```python
from build123d import *

# Parameters (mm, degrees)
BOSS_EXTRUDE1_DEPTH = 16
SKETCH2_R           = 1
CUT_EXTRUDE1_DEPTH  = 16


with BuildPart() as part:
    # Sketch1 → Boss-Extrude1 (new body)
    with BuildSketch(Plane.XY):
        with BuildLine():
            Line((0, 0), (4, 0))
            ThreePointArc((4, 0), (5.414213562, 0.585786438), (6, 2))
            Line((6, 2), (6, 38))
            ThreePointArc((6, 38), (6.585786438, 39.414213562), (8, 40))
            Line((8, 40), (44, 40))
            ThreePointArc((44, 40), (45.414213562, 39.414213562), (46, 38))
            Line((46, 38), (46, 2))
            ThreePointArc((46, 2), (46.585786438, 0.585786438), (48, 0))
            Line((48, 0), (52, 0))
            Line((52, 0), (52, 1.5))
            Line((52, 1.5), (48, 1.5))
            ThreePointArc((48, 1.5), (47.646446609, 1.646446609), (47.5, 2))
            Line((47.5, 2), (47.5, 38))
            ThreePointArc((47.5, 38), (46.474873734, 40.474873734), (44, 41.5))
            Line((44, 41.5), (8, 41.5))
            ThreePointArc((8, 41.5), (5.525126266, 40.474873734), (4.5, 38))
            Line((4.5, 38), (4.5, 2))
            ThreePointArc((4.5, 2), (4.353553391, 1.646446609), (4, 1.5))
            Line((4, 1.5), (0, 1.5))
            Line((0, 1.5), (0, 0))
        make_face()
    extrude(amount=BOSS_EXTRUDE1_DEPTH)

    # Sketch2 → Cut-Extrude1 (cut)
    with BuildSketch(Plane(origin=(0, 1.5, 0), x_dir=(1, 0, 0), z_dir=(0, 1, 0))):
        with Locations(Location((50, -3, 0), (0, 0, 180))):
            Circle(SKETCH2_R)
        with Locations(Location((50, -13, 0), (0, 0, 180))):
            Circle(SKETCH2_R)
        with Locations(Location((2, -3, 0), (0, 0, 180))):
            Circle(SKETCH2_R)
        with Locations(Location((2, -13, 0), (0, 0, 180))):
            Circle(SKETCH2_R)
    extrude(amount=-CUT_EXTRUDE1_DEPTH, mode=Mode.SUBTRACT)


solid = part.part
```
Design review of the part built by this model. Coordinates are the model's own, in mm. A direction names the side the tool comes from. Coordinates: 2 decimals unless noted, no trailing zeros. Loops run counter-clockwise (first coordinate to the right, second up) from the corner with the lowest first, then second, coordinate; pieces in that order, holes last. Notation, with made-up numbers: (48, 78.25) -> (66, 78.25) arc R21 ccw to (66, 110.25) -> close; hole circle Ø1 at (68.5, -18.75). An arc over 180 degrees is marked (long way). Answer as a JSON object with one key per item and string values.
Q1. Clearance check with flat-ended pins moving along their axes: pin 1 Ø3 at (y, z) = (9, 11) entering from +X; pin 2 Ø6 at (x, z) = (5.5, 4) entering from +Y; pin 3 Ø2 at (x, z) = (1.5, 4.5) entering from +Y; pin 4 Ø5 at (x, z) = (26.5, 11) entering from -Y. State where each tip first meets the part, or that it passes through.
Answer block:
{"pin 1": "stops at x = 47.5", "pin 2": "stops at y = 41.5", "pin 3": "stops at y = 1.5", "pin 4": "stops at y = 40"}
Q2. Take a section at B-B on x = 2. Give the boundary of the cut face in (y, z), plus the area to 3 significant figures.
Answer block:
{"outline": "(0, 0) -> (1.5, 0) -> (1.5, 2) -> (0, 2) -> close; (0, 4) -> (1.5, 4) -> (1.5, 12) -> (0, 12) -> close; (0, 14) -> (1.5, 14) -> (1.5, 16) -> (0, 16) -> close", "area": "18.0 mm^2"}
Q3. Take a section at A-A on y = 5. Give the boundary of the cut face in (x, z), plus the area to 3 significant figures.
Answer block:
{"outline": "(4.5, 0) -> (6, 0) -> (6, 16) -> (4.5, 16) -> close; (46, 0) -> (47.5, 0) -> (47.5, 16) -> (46, 16) -> close", "area": "48.0 mm^2"}
Q4. Tool access review of faces 4 (the flat face through (50, 1.5, 8)), 5 (the flat face through (4.5, 20, 8)), 6 (the cylindrical face through (46.57, 0.6, 7.89)): name each direction out of +Z, -Z, +X, -X, +Y, -Y from which nothing blocks a thin tool from reaching the whole face with its end or side.
Answer block:
{"face 4": "+Z, -Z, +X, +Y", "face 5": "+Z, -Z, -X, +Y", "face 6": "+Z, -Z, -Y"}
Q5. Take a section at C-C on z = 3. Give the boundary of the cut face in (x, y), plus the area to 3 significant figures.
Answer block:
{"outline": "(0, 0) -> (1, 0) -> (1, 1.5) -> (0, 1.5) -> close; (3, 0) -> (4, 0) arc R2 ccw to (6, 2) -> (6, 38) arc R2 cw to (8, 40) -> (44, 40) arc R2 cw to (46, 38) -> (46, 2) arc R2 ccw to (48, 0) -> (49, 0) -> (49, 1.5) -> (48, 1.5) arc R0.5 cw to (47.5, 2) -> (47.5, 38) arc R3.5 ccw to (44, 41.5) -> (8, 41.5) arc R3.5 ccw to (4.5, 38) -> (4.5, 2) arc R0.5 cw to (4, 1.5) -> (3, 1.5) -> close; (51, 0) -> (52, 0) -> (52, 1.5) -> (51, 1.5) -> close", "area": "187 mm^2"}
Q6. To check wall thickness, follow L1, parallel to Z at x = 2, y = 1.25; L2, parallel to X at y = 13.5, z = 11.75; L3, parallel to Y at x = 37, z = 11.25. State the ranges of each line that lie inside material, in increasing order.
Answer block:
{"L1": "z = 0 to 2, 4 to 12, 14 to 16", "L2": "x = 4.5 to 6, 46 to 47.5", "L3": "y = 40 to 41.5"}
Q7. The part is to be moulded in two halves that separate along Z. For faces 1 (the cylindrical face through (49, 1, 13)), 2 (the flat face through (26, 41, 0)), 3 (the flat face through (52, 1, 8)), say which applies: +Z half, -Z half, draft (parallel to the pull), parting line (faces both ways), or undercut.
Answer block:
{"face 1": "undercut", "face 2": "-Z half", "face 3": "draft"}
Q8. Take a section at D-D on z = 8.75. Give the boundary of the cut face in (x, y), plus the area to 3 significant figures.
Answer block:
{"outline": "(0, 0) -> (4, 0) arc R2 ccw to (6, 2) -> (6, 38) arc R2 cw to (8, 40) -> (44, 40) arc R2 cw to (46, 38) -> (46, 2) arc R2 ccw to (48, 0) -> (52, 0) -> (52, 1.5) -> (48, 1.5) arc R0.5 cw to (47.5, 2) -> (47.5, 38) arc R3.5 ccw to (44, 41.5) -> (8, 41.5) arc R3.5 ccw to (4.5, 38) -> (4.5, 2) arc R0.5 cw to (4, 1.5) -> (0, 1.5) -> close", "area": "193 mm^2"}
